Can you work these out from the model? Positions are in its coordinate system, mm. A direction names the side the tool comes from. Coordinates: 2 decimals unless noted, no trailing zeros. Loops run counter-clockwise (first coordinate to the right, second up) from the corner with the lowest first, then second, coordinate; pieces in that order, holes last.
```python
from build123d import *

# Parameters (mm, degrees)
BRACKET_PROFILE_SKETCH_R   = 15
BRACKET_PROFILE_SKETCH_R_2 = 9
BRACKET_BODY_DEPTH         = 85
GUSSET_TRIM_SKETCH_W       = 152.495630812
GUSSET_TRIM_SKETCH_H       = 155.202581702
GUSSET_TRIM_CUT_DEPTH      = 73
BASE_GROOVE_SKETCH_W       = 49
BASE_GROOVE_SKETCH_H       = 3
BASE_GROOVE_DEPTH          = 202.86381548
PIVOT_BOSSES_SKETCH_R      = 15
PIVOT_BOSS_36MM_DEPTH      = 18
SKETCH13_3_R               = 9
PIVOT_BOSS_30MM_DEPTH      = 30
MOUNTING_HOLES_SKETCH_R    = 8
BASE_MOUNTING_HOLES_DEPTH  = 30


with BuildPart() as part:
    # Bracket Profile Sketch → Bracket Body (new body)
    with BuildSketch(Plane.XY):
        with BuildLine():
            Line((-90, -62), (-90, -118))
            Line((-90, -118), (50, -118))
            Line((50, -118), (50, -100))
            Line((50, -100), (26.866088482, 5.870544241))
            ThreePointArc((26.866088482, 5.870544241), (-2.952335241, 27.341062829), (-27.5, 0))
            Line((-27.5, 0), (-27.5, -17))
            ThreePointArc((-27.5, -17), (-34.82233047, -34.67766953), (-52.5, -42))
            Line((-52.5, -42), (-70, -42))
            ThreePointArc((-70, -42), (-84.142135624, -47.857864376), (-90, -62))
        make_face()
        Circle(BRACKET_PROFILE_SKETCH_R, mode=Mode.SUBTRACT)
        with Locations((-70, -62)):
            Circle(BRACKET_PROFILE_SKETCH_R_2, mode=Mode.SUBTRACT)
    extrude(amount=BRACKET_BODY_DEPTH)

    # Gusset Trim Sketch → Gusset Trim Cut (cut)
    with BuildSketch(Plane.XY.offset(85)):
        with Locations((-26.247815406, -22.398709149)):
            Rectangle(GUSSET_TRIM_SKETCH_W, GUSSET_TRIM_SKETCH_H)
    extrude(amount=-GUSSET_TRIM_CUT_DEPTH, mode=Mode.SUBTRACT)

    # Base Groove Sketch → Base Groove (cut, through all)
    with BuildSketch(Plane.ZY.offset(90)):
        with Locations((44.711476451, -116.5)):
            Rectangle(BASE_GROOVE_SKETCH_W, BASE_GROOVE_SKETCH_H)
    extrude(amount=-BASE_GROOVE_DEPTH, mode=Mode.SUBTRACT)

    # Pivot Bosses Sketch → Pivot Boss 36mm (add, symmetric)
    with BuildSketch(Plane.XY.offset(12)):
        with BuildLine():
            ThreePointArc((-27.5, 0), (0, -27.5), (27.5, 0))
            ThreePointArc((27.5, 0), (27.341062829, 2.952335241), (26.866088482, 5.870544241))
            ThreePointArc((26.866088482, 5.870544241), (-2.952335241, 27.341062829), (-27.5, 0))
        make_face()
        Circle(PIVOT_BOSSES_SKETCH_R, mode=Mode.SUBTRACT)
    extrude(amount=PIVOT_BOSS_36MM_DEPTH, both=True)

    # Sketch13_3 → Pivot Boss 30mm (add)
    with BuildSketch(Plane.XY.offset(12)):
        with BuildLine():
            ThreePointArc((-90, -62), (-70, -82), (-50, -62))
            ThreePointArc((-50, -62), (-55.857864376, -47.857864376), (-70, -42))
            ThreePointArc((-70, -42), (-84.142135624, -47.857864376), (-90, -62))
        make_face()
        with Locations((-70, -62)):
            Circle(SKETCH13_3_R, mode=Mode.SUBTRACT)
    extrude(amount=PIVOT_BOSS_30MM_DEPTH)

    # Mounting Holes Sketch → Base Mounting Holes (cut)
    with BuildSketch(Plane(origin=(0, -100, 0), x_dir=(1, 0, 0), z_dir=(0, 1, 0))):
        with Locations(Location((-55, -55, 0), (0, 0, 180))):
            Circle(MOUNTING_HOLES_SKETCH_R)
        with Locations(Location((15, -55, 0), (0, 0, 180))):
            Circle(MOUNTING_HOLES_SKETCH_R)
    extrude(amount=-BASE_MOUNTING_HOLES_DEPTH, mode=Mode.SUBTRACT)


solid = part.part
```
(1) I want a section at A-A on z = 18. Write out the boundary of the cut face in (x, y), then the cut area to 3 significant figures.
Check values:
outline: (-90, -118) - (50, -118) - (50, -100) - (-90, -100) - close; circle Ø40 at (-70, -62); circle Ø55 at (0, 0); hole circle Ø18 at (-70, -62); hole circle Ø30 at (0, 0)
area: 5,190 mm2
(2) I want a section at B-B on x = 0. Write out the boundary of the cut face in (y, z).
Check values:
outline: (-118, 0) - (-27.5, 0) - (-27.5, -6) - (-15, -6) - (-15, 30) - (-27.5, 30) - (-27.5, 12) - (-100, 12) - (-100, 85) - (-118, 85) - (-118, 69.21) - (-115, 69.21) - (-115, 20.21) - (-118, 20.21) - close; (15, -6) - (27.5, -6) - (27.5, 30) - (15, 30) - close
(3) I'm going to push flat-ended pins straight in: pin 1 (8 mm diameter, centred on x = -21.5, y = -91, fed in from -Z); pin 2 (10 mm diameter, centred on x = 26.5, z = 42.5, fed in from +Y); pin 3 (23.5 mm diameter, centred on x = -70, y = -62, fed in from +Z). Where does each tip first touch, or does it pass through?
Check values:
pin 1: stops at z = 0
pin 2: stops at y = -100
pin 3: stops at z = 42
(4) If I drill on probe 1 along Y at (x, z) = (0, 22.25); probe 2 along Y at (x, z) = (-74.5, 28.5); probe 3 along Z at (x, y) = (-22.5, -30), over which ranges is the centre line in solid material (lowest first)?
Check values:
probe 1: y = -115 to -100, -27.5 to -15, 15 to 27.5
probe 2: y = -115 to -100, -81.49 to -69.79, -54.21 to -42.51
probe 3: z = 0 to 12
(5) I want a section at D-D on y = -108. Write out the boundary of the cut face in (x, z).
Check values:
outline: (-90, 0) - (50, 0) - (50, 85) - (-90, 85) - close; hole circle Ø16 at (-55, 55); hole circle Ø16 at (15, 55)
(6) If we mould it in two halves opening along Z, with no side actions, what happens to faces 1 (the cylindrical face through (-61.686, -65.447, 20.706)), 2 (the cylindrical face through (-49.1, -107.4, 60.4)), 3 (the flat face through (12, -12, 30))? For each: released by +Z, released by -Z, zero draft, split by the parting line, or undercut.
Check values:
face 1: zero draft
face 2: undercut
face 3: released by +Z
(7) Which directions (+Z, -Z, +X, -X, +Y, -Y) give clear straight access to the entire face, cutting with the end or side of a thin tool? Please do faces 4 (the flat face through (-21, -115, 44)), 5 (the flat face through (-21, -100, 49)), 6 (the flat face through (-66, -71, 42)), 7 (the flat face through (-27.5, -8, 6)).
Check values:
face 4: +X, -X, -Y
face 5: +Z, +X, -X
face 6: +Z, +X, -X, +Y
face 7: +Z, -Z, -X, +Y
(8) I want a section at C-C on z = 55. Write out the boundary of the cut face in (x, y), then the cut area to 3 significant figures.
Check values:
outline: (-90, -115) - (-63, -115) - (-63, -100) - (-90, -100) - close; (-47, -115) - (7, -115) - (7, -100) - (-47, -100) - close; (23, -115) - (50, -115) - (50, -100) - (23, -100) - close
area: 1,620 mm2
